Source: CAD feature listing. Evaluate the final solid. Frame: model axes, mm. Give positions to 0.01 mm unless a question says otherwise; leave off trailing zeros. Order: outer loops, then holes, each group sorted by start corner. A loop starts at its lowest first (then second) coordinate and runs counter-clockwise, first axis right, second up.
from build123d import *

# Parameters (mm, degrees)
EXTRUDE_1_DEPTH              = 3
HOLE_WIZARD_M4_1_D           = 4.5
HOLE_WIZARD_M4_1_DEPTH       = 10.1
HOLE_WIZARD_M4_1_CSINK_D     = 9.4
HOLE_WIZARD_M4_1_CSINK_ANGLE = 90
HOLE_WIZARD_M4_1_TIP         = 1.351936393
SKETCH_4_R                   = 47.5
CUT_EXTRUDE_1_DEPTH          = 12
SKETCH_5_R                   = 50
SKETCH_5_R_2                 = 48.5
CUT_EXTRUDE_2_DEPTH          = 1.2
SKETCH_6_R                   = 2.25
CUT_EXTRUDE_3_DEPTH          = 10


with BuildPart() as part:
    # 草图1 → 凸台-拉伸1 (new body)
    with BuildSketch(Plane.XY):
        with BuildLine():
            Line((227.012333385, 39.0187092), (227.012333385, 584.0187092))
            ThreePointArc((227.012333385, 584.0187092), (223.35116815, 592.857543965), (214.512333385, 596.5187092))
            Line((214.512333385, 596.5187092), (-460.487666615, 596.5187092))
            ThreePointArc((-460.487666615, 596.5187092), (-469.326501379, 592.857543965), (-472.987666615, 584.0187092))
            Line((-472.987666615, 584.0187092), (-472.987666615, 39.0187092))
            ThreePointArc((-472.987666615, 39.0187092), (-469.326501379, 30.179874435), (-460.487666615, 26.5187092))
            Line((-460.487666615, 26.5187092), (214.512333385, 26.5187092))
            ThreePointArc((214.512333385, 26.5187092), (223.35116815, 30.179874435), (227.012333385, 39.0187092))
        make_face()
    extrude(amount=EXTRUDE_1_DEPTH)

    # M4 锥坑平头螺钉的锥形沉头孔1
    with Locations(Plane.XY.offset(3)):
        with Locations((222.012333385, 71.5187092), (222.012333385, 191.5187092), (222.012333385, 311.5187092), (222.012333385, 431.5187092), (222.012333385, 551.5187092), (167.012333385, 591.5187092), (22.012333385, 591.5187092), (-122.987666615, 591.5187092), (-267.987666615, 591.5187092), (-412.987666615, 591.5187092), (-467.987666615, 551.5187092), (-467.987666615, 431.5187092), (-467.987666615, 311.5187092), (-467.987666615, 191.5187092), (-467.987666615, 71.5187092), (-412.987666615, 31.5187092), (-267.987666615, 31.5187092), (-122.987666615, 31.5187092), (22.012333385, 31.5187092), (167.012333385, 31.5187092)):
            CounterSinkHole(HOLE_WIZARD_M4_1_D / 2, HOLE_WIZARD_M4_1_CSINK_D / 2, depth=HOLE_WIZARD_M4_1_DEPTH, counter_sink_angle=HOLE_WIZARD_M4_1_CSINK_ANGLE)
            with Locations((0, 0, -(HOLE_WIZARD_M4_1_DEPTH + HOLE_WIZARD_M4_1_TIP / 2))):  # 118° drill point
                Cone(0, HOLE_WIZARD_M4_1_D / 2, HOLE_WIZARD_M4_1_TIP, mode=Mode.SUBTRACT)

    # 草图4 → 切除-拉伸1 (cut)
    with BuildSketch(Plane.XY.offset(3)):
        with Locations((27.012333385, 311.5187092)):
            Circle(SKETCH_4_R)
    extrude(amount=-CUT_EXTRUDE_1_DEPTH, mode=Mode.SUBTRACT)

    # 草图5 → 切除-拉伸2 (cut)
    with BuildSketch(Plane.XY.offset(3)):
        with Locations((27.012333385, 311.5187092)):
            Circle(SKETCH_5_R)
        with Locations((27.012333385, 311.5187092)):
            Circle(SKETCH_5_R_2, mode=Mode.SUBTRACT)
    extrude(amount=-CUT_EXTRUDE_2_DEPTH, mode=Mode.SUBTRACT)

    # 草图6 → 切除-拉伸3 (cut)
    with BuildSketch(Plane.XY.offset(3)):
        with Locations((27.012333385, 258.5187092)):
            Circle(SKETCH_6_R)
        with Locations((-10.464326017, 274.042049797)):
            Circle(SKETCH_6_R)
        with Locations((-25.987666615, 311.5187092)):
            Circle(SKETCH_6_R)
        with Locations((-10.464326017, 348.995368603)):
            Circle(SKETCH_6_R)
        with Locations((27.012333385, 364.5187092)):
            Circle(SKETCH_6_R)
        with Locations((64.488992788, 348.995368603)):
            Circle(SKETCH_6_R)
        with Locations((80.012333385, 311.5187092)):
            Circle(SKETCH_6_R)
        with Locations((64.488992788, 274.042049797)):
            Circle(SKETCH_6_R)
    extrude(amount=-CUT_EXTRUDE_3_DEPTH, mode=Mode.SUBTRACT)


solid = part.part
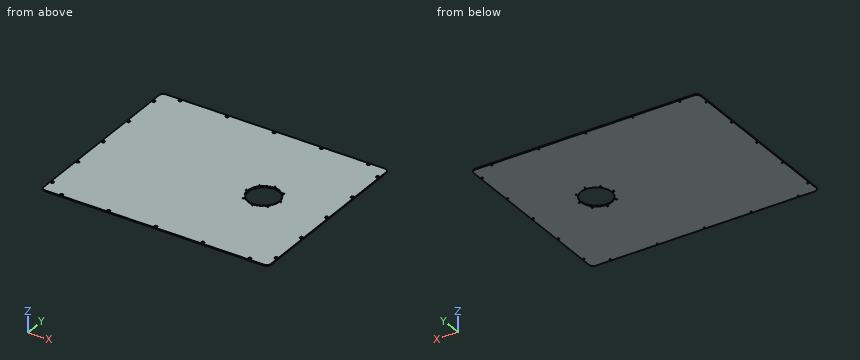
1) Section query C-C on z = 1.05. State how many separate pieces and enclosed holes the cut face has, and give its area (3 significant figures).
Checks:
separate pieces: 1
enclosed holes: 29
area: 391,000 mm2
2) Section query B-B on y = 328. Output: boundary loops of the cut face in (x, z).
Checks:
outline: (-472.99, 0) - (-17.54, 0) - (-17.54, 3) - (-18.6, 3) - (-18.6, 1.8) - (-20.19, 1.8) - (-20.19, 3) - (-472.99, 3) - close; (71.56, 0) - (227.01, 0) - (227.01, 3) - (74.22, 3) - (74.22, 1.8) - (72.63, 1.8) - (72.63, 3) - (71.56, 3) - close
3) Section query A-A on x = 52. Output: boundary loops of the cut face in (y, z).
Checks:
outline: (26.52, 0) - (271.12, 0) - (271.12, 3) - (269.95, 3) - (269.95, 1.8) - (268.21, 1.8) - (268.21, 3) - (26.52, 3) - close; (351.92, 0) - (596.52, 0) - (596.52, 3) - (354.83, 3) - (354.83, 1.8) - (353.09, 1.8) - (353.09, 3) - (351.92, 3) - close
4) First-contact query: pin 1 Ø2.5 at (x, y) = (-467.99, 71.52) entering from -Z; pin 2 Ø5 at (x, y) = (-467.99, 191.52) entering from +Z. Flat tips, straight axial feed; report the tip coordinate or a pass-through.
Checks:
pin 1: passes through
pin 2: stops at z = 0.8
5) Ray query, L1, parallel to X at y = 335, z = 2.3; L2, parallel to Y at x = 15.5, z = 1.9; L3, parallel to X at y = 280, z = 0.7. Return the intervals inside material, ascending.
Checks:
L1: x = -472.99 to -17.13, -15.42 to -14.28, 68.3 to 69.45, 71.16 to 227.01
L2: y = 26.52 to 262.86, 264.4 to 265.43, 357.6 to 358.63, 360.18 to 596.52
L3: x = -472.99 to -8.52, 62.55 to 227.01
